from build123d import *

# Parameters (mm, degrees)
SKETCH_1_R      = 10
EXTRUDE_1_DEPTH = 8


with BuildPart() as part:
    # 草图1 → 凸台-拉伸1 (new body)
    with BuildSketch(Plane.XY):
        with BuildLine():
            Line((0, 0), (80, 0))
            Line((80, 0), (64.318869123, 65.795912749))
            ThreePointArc((64.318869123, 65.795912749), (40, 85), (15.681130877, 65.795912749))
            Line((15.681130877, 65.795912749), (0, 0))
        make_face()
        with Locations((40, 60)):
            Circle(SKETCH_1_R, mode=Mode.SUBTRACT)
    extrude(amount=EXTRUDE_1_DEPTH)


solid = part.part
Source: CAD feature listing. Evaluate the final solid. Frame: model axes, mm. Round coordinates to 2 decimals unless told otherwise and drop trailing zeros. Loops run counter-clockwise (first coordinate to the right, second up) from the corner with the lowest first, then second, coordinate; pieces in that order, holes last. Notation, with made-up numbers: (74.5, 55) - (84.5, 55) arc R16 cw to (84.5, 75) - close; hole circle Ø1 at (45.5, -18). An arc over 180 degrees is marked (long way). Write item = value, one per line. Start each with the question number.
Item 1: Section query A-A on x = 40. Output: boundary loops of the cut face in (y, z).
Item 2: Material intervals for line 1 (Y direction, x = 40, z = 5.5); line 2 (X direction, y = 51, z = 1.75); line 3 (Y direction, x = 39, z = 1.25), sorted ascending.
Item 3: Mould query, pull axis X, two halves, no side actions, for faces 1 (the face through (7.95, 33.36, 3.94)), 2 (the face through (39, 34, 0)), 3 (the face through (37.83, 50.24, 3.94)). Classes: released by +X, released by -X, zero draft, split by the parting line, or undercut.
Item 4: Section query D-D on y = 28. Output: boundary loops of the cut face in (x, z).
Item 5: Section query C-C on z = 5. Output: boundary loops of the cut face in (x, y), plus the area to 3 significant figures.
Item 6: Section query B-B on y = 61.5. Output: boundary loops of the cut face in (x, z).
Results list:
q1.outline = (0, 0) - (50, 0) - (50, 8) - (0, 8) - close; (70, 0) - (85, 0) - (85, 8) - (70, 8) - close
q2.line_1 = 0 to 50, 70 to 85
q2.line_2 = 12.15 to 35.64, 44.36 to 67.85
q2.line_3 = 0 to 50.05, 69.95 to 84.98
q3.face_1 = released by -X
q3.face_2 = zero draft
q3.face_3 = undercut
q4.outline = (6.67, 0) - (73.33, 0) - (73.33, 8) - (6.67, 8) - close
q5.outline = (0, 0) - (80, 0) - (64.32, 65.8) arc R25 ccw to (15.68, 65.8) - close; hole circle Ø20 at (40, 60)
q5.area = 4,610 mm²
q6.outline = (14.66, 0) - (30.11, 0) - (30.11, 8) - (14.66, 8) - close; (49.89, 0) - (65.34, 0) - (65.34, 8) - (49.89, 8) - close
